```python
from build123d import *

# Parameters (mm, degrees)
SKETCH_1_W          = 25.5
SKETCH_1_H          = 40
EXTRUDE_1_DEPTH     = 6.5
SKETCH_2_R          = 6
EXTRUDE_2_DEPTH     = 40
SKETCH_3_W          = 27
SKETCH_3_H          = 25
CUT_EXTRUDE_1_DEPTH = 30.925950277
SKETCH_5_R          = 3.5
CUT_EXTRUDE_2_DEPTH = 29.174678348
CHAMFER_1_SIZE      = 3


with BuildPart() as part:
    # 草图1 → 凸台-拉伸1 (new body)
    with BuildSketch(Plane(origin=(0, 0, 0), x_dir=(1, 0, 0), z_dir=(0, 1, 0))):
        Rectangle(SKETCH_1_W, SKETCH_1_H)
    extrude(amount=EXTRUDE_1_DEPTH)

    # 草图2 → 凸台-拉伸2 (add)
    with BuildSketch(Plane.XY.offset(20)):
        with Locations((12.75, 6)):
            Circle(SKETCH_2_R)
    extrude(amount=-EXTRUDE_2_DEPTH)

    # 草图3 → 切除-拉伸1 (cut, through all)
    with BuildSketch(Plane.XZ):
        with Locations((18.75, 0)):
            Rectangle(SKETCH_3_W, SKETCH_3_H)
    extrude(amount=-CUT_EXTRUDE_1_DEPTH, mode=Mode.SUBTRACT)

    # 草图5 → 切除-拉伸2 (cut, through all)
    with BuildSketch(Plane(origin=(0, 6.5, 0), x_dir=(1, 0, 0), z_dir=(0, 1, 0))):
        with Locations(Location((-2.25, 12, 0), (0, 0, 270))):
            Circle(SKETCH_5_R)
        with Locations(Location((-2.25, -12, 0), (0, 0, 270))):
            Circle(SKETCH_5_R)
    extrude(amount=-CUT_EXTRUDE_2_DEPTH, mode=Mode.SUBTRACT)

    # 倒角1
    chamfer_1_edges = [part.edges().sort_by_distance(p)[0] for p in [
        (-2.25, 6.5, -15.5),
        (-2.25, 6.5, 8.5),
    ]]
    chamfer(chamfer_1_edges, length=CHAMFER_1_SIZE)


solid = part.part
```
Input: part model. Units: mm. Frame: model coordinates. A direction names the side the tool comes from. Give positions to 0.01 mm unless a question says otherwise; leave off trailing zeros. Order: outer loops, then holes, each group sorted by start corner. A loop starts at its lowest first (then second) coordinate and runs counter-clockwise, first axis right, second up. Notation, with made-up numbers: (20, 10.5) -> (48, 10.5) arc R32 ccw to (48, 43.5) -> close; hole circle Ø9 at (87, -6.75). An arc over 180 degrees is marked (long way). Write each question's results on one line, items separated by ' | '. Start each with the question number.
Item 1: Cut plane D-D on x = 9.5. Return the cut outline in (y, z).
Item 2: Mould query, pull axis Z, two halves, no side actions, for faces 1 (the flat face through (3, 5, -20)), 2 (the cylindrical face through (-2.096, 1.774, -15.497)), 3 (the flat face through (5.25, 3, 0)), 4 (the cylindrical face through (17.295, 9.917, -16.197)). Classes: pulls with the +Z half, pulls with the -Z half, needs draft (parallel to the pull), parting line crosses it, or undercut.
Item 3: Cut plane A-A on z = 12. Return the cut outline in (x, y), then the cut area to 3 significant figures.
Item 4: Cut plane B-B on x = -2.25. Return the cut outline in (y, z), then the cut area to 3 significant figures.
Item 5: Line query: line 1 (Z direction, x = 15.5, y = 3); line 2 (Z direction, x = -4, y = 1.5); line 3 (X direction, y = 1.15, z = 12). Output: solid intervals per line, ascending.
Item 6: Contact query for flat-ended pins moving along their axis: P1, Ø3, axis at x = -2.5, z = -8, coming from the +Y side; P2, Ø3, axis at y = 7.5, z = -2.5, coming from the -X side; P3, Ø15.5, axis at x = -1, z = -1.5, coming from the +Y side; P4, Ø2, axis at y = 4, z = 1.5, coming from the +X side. Output: stop coordinate, or through.
Item 7: Set-up query: faces 5 (the flat face through (-5, 6.5, 0)), 6 (the conical face through (-1.15, 3.65, 15.48)), 7 (the flat face through (12, 6, 12.5)). Return all of +Z, -Z, +X, -X, +Y, -Y with unobstructed straight access to the full face (end or side cutting, diameter ignored); none if empty.
Item 8: Cut plane C-C on y = 8.25. Return the cut outline in (x, z), then the cut area to 3 significant figures.
Established:
1) outline: (0, -20) -> (11.04, -20) -> (11.04, -12.5) -> (0, -12.5) -> close; (0, 12.5) -> (11.04, 12.5) -> (11.04, 20) -> (0, 20) -> close
2) face 1: pulls with the -Z half | face 2: undercut | face 3: undercut | face 4: needs draft
3) outline: (-12.75, 0) -> (-5.75, 0) -> (-5.75, 3.5) -> (-8.75, 6.5) -> (-12.75, 6.5) -> close; (1.25, 0) -> (5.25, 0) -> (5.25, 6.5) -> (4.25, 6.5) -> (1.25, 3.5) -> close | area: 62.5 mm^2
4) outline: (0, -20) -> (6.5, -20) -> (6.5, -18.5) -> (3.5, -15.5) -> (0, -15.5) -> close; (0, -8.5) -> (3.5, -8.5) -> (6.5, -5.5) -> (6.5, 5.5) -> (3.5, 8.5) -> (0, 8.5) -> close; (0, 15.5) -> (3.5, 15.5) -> (6.5, 18.5) -> (6.5, 20) -> (0, 20) -> close | area: 151 mm^2
5) line 1: -20 to -12.5, 12.5 to 20 | line 2: -20 to -15.03, -8.97 to 8.97, 15.03 to 20 | line 3: -12.75 to -5.75, 1.25 to 5.25
6) P1: y = 5.51 | P2: x = -12.75 | P3: y = 6.5 | P4: x = 5.25
7) face 5: +Z, -Z, -X, +Y | face 6: +Y | face 7: +X, +Y, -Y
8) outline: (7.19, -20) -> (18.31, -20) -> (18.31, -12.5) -> (7.19, -12.5) -> close; (7.19, 12.5) -> (18.31, 12.5) -> (18.31, 20) -> (7.19, 20) -> close | area: 167 mm^2
